```python
from build123d import *

# Parameters (mm, degrees)
SKETCH_1_R      = 25
EXTRUDE_1_DEPTH = 100
SKETCH_2_R      = 7.5
EXTRUDE_2_DEPTH = 10
EXTRUDE_START   = 80
SKETCH_3_R      = 7.5
EXTRUDE_3_DEPTH = 80


with BuildPart() as part:
    # 草图1 → 凸台-拉伸1 (new body)
    with BuildSketch(Plane.XY):
        Circle(SKETCH_1_R)
    extrude(amount=EXTRUDE_1_DEPTH)

    # 草图2 → 凸台-拉伸2 (add)
    with BuildSketch(Plane.XY.offset(100)):
        Circle(SKETCH_2_R)
    extrude(amount=EXTRUDE_2_DEPTH)

    # 草图3 → 凸台-拉伸3 (add)
    with BuildSketch(Plane(origin=(0, 0, 0), x_dir=(-1, 0, 0), z_dir=(0, 0, -1)).offset(EXTRUDE_START)):
        with Locations(Location((0, 0, 0), (0, 0, 180))):
            Circle(SKETCH_3_R)
    extrude(amount=-EXTRUDE_3_DEPTH)


solid = part.part
```
Read the model definition and answer for the solid it produces. Units are mm, in the model's axes. A direction names the side the tool comes from. Coordinates: 2 decimals unless noted, no trailing zeros. Write each loop counter-clockwise with the first axis right and the second up, starting at its lowest first coordinate (ties: lowest second). Pieces come first, ordered by that corner, then holes. Notation, with made-up numbers: (6.25, 69.5) -> (34.25, 69.5) arc R24 cw to (34.25, 80.5) -> close; hole circle Ø5 at (25, -16). An arc over 180 degrees is marked (long way). Return JSON: item names as keys, results as strings.
1. Find the intervals of material crossed by line 1 along Z through (x, y) = (-16.5, -8); line 2 along X through (y, z) = (-23, 18.5); line 3 along Y through (x, z) = (15, 98.5), in increasing order. Write a range as from..to.
Found:
{"line 1": "0..100", "line 2": "-9.8..9.8", "line 3": "-20..20"}
2. A cutting plane is placed at D-D (z = -9). Determine the outline of the cut face in (x, y), and give its area (3 significant figures).
Found:
{"outline": "circle Ø15 at (0, 0)", "area": "177 mm2"}
3. A cutting plane is placed at C-C (z = 22). Determine the outline of the cut face in (x, y), and give its area (3 significant figures).
Found:
{"outline": "circle Ø50 at (0, 0)", "area": "1,960 mm2"}
4. A cutting plane is placed at A-A (x = 0). Determine the outline of the cut face in (y, z).
Found:
{"outline": "(-25, 0) -> (-7.5, 0) -> (-7.5, -80) -> (7.5, -80) -> (7.5, 0) -> (25, 0) -> (25, 100) -> (7.5, 100) -> (7.5, 110) -> (-7.5, 110) -> (-7.5, 100) -> (-25, 100) -> close"}
5. Each of these flat-tipped pins is pushed along its axis until it touches: P1, Ø1, axis at x = -4, z = 89.5, coming from the -Y side; P2, Ø5, axis at x = -2, z = 73, coming from the -Y side; P3, Ø4, axis at x = 12, y = 6, coming from the -Z side; P4, Ø25, axis at x = 8.5, y = -4.5, coming from the +Z side. Where does it stop, or does it pass through?
Found:
{"P1": "y = -24.75", "P2": "y = -25", "P3": "z = 0", "P4": "z = 110"}
6. A tool of negligible diameter and unlimited length cuts with its end or side. For faces 1 (the face through (0, 0, 110)), 2 (the face through (-6, -5, 100)), 3 (the face through (-6, -5, 0)), from which of +Z, -Z, +X, -X, +Y, -Y can it reach the whole face along a straight path? Write none if from no direction.
Found:
{"face 1": "+Z, +X, -X, +Y, -Y", "face 2": "+Z", "face 3": "-Z"}
